Input: part model. Units: mm. Frame: model coordinates. A direction names the side the tool comes from. Give positions to 0.01 mm unless a question says otherwise; leave off trailing zeros. Order: outer loops, then holes, each group sorted by start corner. A loop starts at its lowest first (then second) coordinate and runs counter-clockwise, first axis right, second up. Notation, with made-up numbers: (3.5, 50) - (56.5, 50) arc R19 ccw to (56.5, 74) - close; hole circle Ø9 at (-33.5, 26.5). An arc over 180 degrees is marked (long way). Answer in a Markdown table with one row per item. Add a question column.
from build123d import *

# Parameters (mm, degrees)
SKETCH1_R           = 6
BOSS_EXTRUDE1_DEPTH = 10
CUT_EXTRUDE1_DEPTH  = 5
CHAMFER1_SIZE       = 1


with BuildPart() as part:
    # Sketch1 → Boss-Extrude1 (new body)
    with BuildSketch(Plane.XY):
        Circle(SKETCH1_R)
    extrude(amount=BOSS_EXTRUDE1_DEPTH)

    # Sketch2 → Cut-Extrude1 (cut)
    with BuildSketch(Plane.XY.offset(10)):
        Polygon((0, 3.129298789), (-2.710052247, 1.564649395), (-2.710052247, -1.564649395), (0, -3.129298789), (2.710052247, -1.564649395), (2.710052247, 1.564649395), align=None)
    extrude(amount=-CUT_EXTRUDE1_DEPTH, mode=Mode.SUBTRACT)

    # Chamfer1
    chamfer1_edges = [part.edges().sort_by_distance(p)[0] for p in [
        (-6, 0, 0),
        (-6, 0, 10),
    ]]
    chamfer(chamfer1_edges, length=CHAMFER1_SIZE)


solid = part.part
Q1. Section C-C, the plane z = 4.5. Return loops of the section in (x, y), then the cut area to 3 significant figures.
Q2. Contact query for flat-ended pins moving along their axis: P1, Ø1, axis at y = 4, z = 7.5, coming from the -X side; P2, Ø1, axis at y = -3.5, z = 9, coming from the +X side; P3, Ø4, axis at x = 4.5, z = 5.5, coming from the -Y side. Output: stop coordinate, or through.
Q3. Section B-B, the plane y = 0. Return loops of the section in (x, z).
Q4. Section A-A, the plane z = 8.75. Return loops of the section in (x, y), then the cut area to 3 significant figures.
Q5. Pull-direction query (X, two-part tool) for faces 1 (the flat face through (0, 0, 0)), 2 (the cylindrical face through (-6, 0, 5)), 3 (the flat face through (-2.71, 0, 8)); classes: +X half, -X half, draft (parallel to the pull), parting line (faces both ways), or undercut.
Q6. Line query: probe 1 along Z at (x, y) = (0, -2.25); probe 2 along Y at (x, z) = (-1.5, 9.25); probe 3 along X at (y, z) = (-1, 7.5). Output: solid intervals per line, ascending.
Q7. Access query for faces 4 (the flat face through (2.2, -2.2, 10)), 5 (the flat face through (0, 0, 5)). Directions: +Z, -Z, +X, -X, +Y, -Y. A direction counts if a zero-diameter tool reaches every point of the face in a straight line with its end or side. Return the directions, or none.
Computed:
| question | item | result |
|---|---|---|
| 1 | outline | circle Ø12 at (0, 0) |
| 1 | area | 113 mm^2 |
| 2 | P1 | stops at x = -4.87 |
| 2 | P2 | stops at x = 5.2 |
| 2 | P3 | stops at y = -5.45 |
| 3 | outline | (-6, 1) - (-5, 0) - (5, 0) - (6, 1) - (6, 9) - (5, 10) - (2.71, 10) - (2.71, 5) - (-2.71, 5) - (-2.71, 10) - (-5, 10) - (-6, 9) - close |
| 4 | outline | circle Ø12 at (0, 0); hole (-2.71, -1.56) - (0, -3.13) - (2.71, -1.56) - (2.71, 1.56) - (0, 3.13) - (-2.71, 1.56) - close |
| 4 | area | 87.7 mm^2 |
| 5 | face 1 | draft |
| 5 | face 2 | parting line |
| 5 | face 3 | undercut |
| 6 | probe 1 | z = 0 to 5 |
| 6 | probe 2 | y = -5.55 to -2.26, 2.26 to 5.55 |
| 6 | probe 3 | x = -5.92 to -2.71, 2.71 to 5.92 |
| 7 | face 4 | +Z, +X, -X, +Y, -Y |
| 7 | face 5 | +Z |
